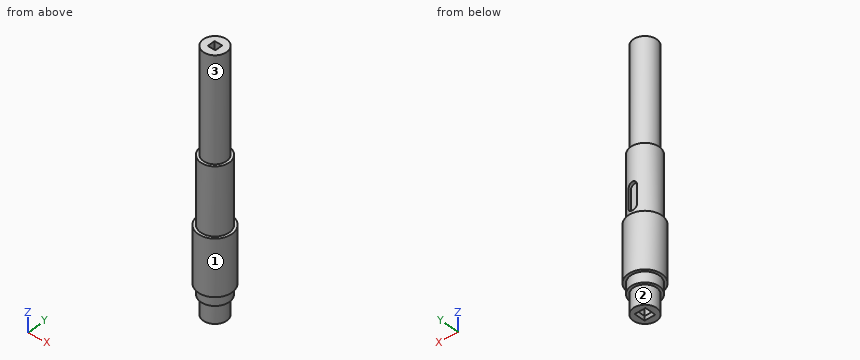
```python
from build123d import *

# Parameters (mm, degrees)
SKETCH_2_W          = 15
SKETCH_2_H          = 15
CUT_EXTRUDE_1_DEPTH = 496.137859591
CHAMFER_1_SIZE      = 3
CHAMFER_1_SIZE2     = 5.196152423
CUT_EXTRUDE_2_DEPTH = 6


with BuildPart() as part:
    # 草图1 → 旋转1 (revolve)
    with BuildSketch(Plane(origin=(0, 0, 0), x_dir=(1, 0, 0), z_dir=(0, 1, 0))):
        Polygon((0, 200), (-22.5, 200), (-22.5, 163), (-27.5, 163), (-27.5, 143), (-32.5, 143), (-32.5, 35.5), (-27.5, 35.5), (-27.5, -93), (-22.5, -93), (-22.5, -293), (0, -293), align=None)
    revolve(axis=Axis((0, 0, 0), (0, 0, 1)))

    # 草图2 → 切除-拉伸1 (cut, through all)
    with BuildSketch(Plane(origin=(0, 0, -200), x_dir=(-1, 0, 0), z_dir=(0, 0, -1))):
        Rectangle(SKETCH_2_W, SKETCH_2_H)
    extrude(amount=-CUT_EXTRUDE_1_DEPTH, mode=Mode.SUBTRACT)

    # 倒角1
    chamfer_1_edges = [part.edges().sort_by_distance(p)[0] for p in [
        (7.5, 0, -200),
        (0, -7.5, -200),
        (-7.5, 0, -200),
        (0, 7.5, -200),
    ]]
    chamfer_1_side = [part.faces().sort_by_distance(p)[0] for p in [
        (21.863603897, 0, -200),
    ]]
    chamfer(chamfer_1_edges, length=CHAMFER_1_SIZE, length2=CHAMFER_1_SIZE2, reference=chamfer_1_side[0])

    # 草图3 → 切除-拉伸2 (cut)
    with BuildSketch(Plane(origin=(0, 27.5, 0), x_dir=(1, 0, 0), z_dir=(0, 1, 0))):
        with BuildLine():
            Line((-8, -19.5), (-8, 17.5))
            ThreePointArc((-8, 17.5), (0, 25.5), (8, 17.5))
            Line((8, 17.5), (8, -19.5))
            ThreePointArc((8, -19.5), (0, -27.5), (-8, -19.5))
        make_face()
    extrude(amount=-CUT_EXTRUDE_2_DEPTH, mode=Mode.SUBTRACT)


solid = part.part
```
The model under review builds one solid part; all positions refer to its coordinate system, in mm. Face numbers are marked on the shaded views. A direction names the side the tool comes from. Round coordinates to 2 decimals unless told otherwise and drop trailing zeros. Loops run counter-clockwise (first coordinate to the right, second up) from the corner with the lowest first, then second, coordinate; pieces in that order, holes last. Notation, with made-up numbers: (65.5, 73.25) -> (95.5, 73.25) arc R14 cw to (95.5, 78.25) -> close; hole circle Ø9 at (72.25, 43). An arc over 180 degrees is marked (long way). Answer as a JSON object with one key per item and string values. Group by question number.
1) We need section B-B on y = 0. Write out the cut boundary in (x, z), then the cut area to 3 significant figures.
2) For line 1 (Y direction, x = -2.5, z = -113); line 2 (Z direction, x = 8.5, y = 28.5); line 3 (X direction, y = 0.5, z = 28), list the stretches that pass through material, from the lowest coordinate up. Write a range as [from, to].
3) We need section A-A on z = -7.5. Write out the cut boundary in (x, y).
4) For pin 1 Ø10 at (x, z) = (-16.5, 198.5) entering from +Y; pin 2 Ø12 at (x, z) = (14.5, -36) entering from -Y; pin 3 Ø2 at (y, z) = (-9.5, 50.5) entering from +X; pin 4 Ø7.5 at (y, z) = (1.5, -40.5) entering from -X, all flat-tipped, find the tip position at first contact; note any pin that passes through.
5) For the marked faces 1, 2 and 3, list the 3-axis set-ups (+Z, -Z, +X, -X, +Y, -Y) from which the entire face can be reached by the end or side of a thin tool; tool diameter is ignored.
6) We need section C-C on z = 244.5. Write out the cut boundary in (x, y).
Result set:
{
 "1": {"outline": "(-32.5, -143) -> (-27.5, -143) -> (-27.5, -163) -> (-22.5, -163) -> (-22.5, -200) -> (-10.5, -200) -> (-7.5, -194.8) -> (-7.5, 293) -> (-22.5, 293) -> (-22.5, 93) -> (-27.5, 93) -> (-27.5, -35.5) -> (-32.5, -35.5) -> close; (7.5, -194.8) -> (10.5, -200) -> (22.5, -200) -> (22.5, -163) -> (27.5, -163) -> (27.5, -143) -> (32.5, -143) -> (32.5, -35.5) -> (27.5, -35.5) -> (27.5, 93) -> (22.5, 93) -> (22.5, 293) -> (7.5, 293) -> close", "area": "18,400 mm²"},
 "2": {"line 1": "[-32.4, -7.5], [7.5, 32.4]", "line 2": "[-143, -35.5]", "line 3": "[-27.5, -7.5], [7.5, 27.5]"},
 "3": {"outline": "(-8, 21.5) -> (-8, 26.31) arc R27.5 ccw (long way) to (8, 26.31) -> (8, 21.5) -> close; hole (-7.5, -7.5) -> (7.5, -7.5) -> (7.5, 7.5) -> (-7.5, 7.5) -> close"},
 "4": {"pin 1": "y = 19.34", "pin 2": "y = -31.37", "pin 3": "x = 26.15", "pin 4": "x = -32.5"},
 "5": {"face 1": "+Z, -Z", "face 2": "-Z", "face 3": "+Z"},
 "6": {"outline": "circle Ø45 at (0, 0); hole (-7.5, -7.5) -> (7.5, -7.5) -> (7.5, 7.5) -> (-7.5, 7.5) -> close"}
}
